```python
from build123d import *

# Parameters (mm, degrees)
SKETCH1_W          = 40
SKETCH1_H          = 30
EXTRUDE1_DEPTH     = 15
SKETCH2_R          = 11
EXTRUDE2_DEPTH     = 10
SKETCH3_R          = 10
EXTRUDE3_DEPTH     = 1
SKETCH4_R          = 17.5
EXTRUDE4_DEPTH     = 8
FILLET1_R          = 2
SKETCH5_OUTSIDE_W  = 56.458
SKETCH5_OUTSIDE_H  = 51.458
SKETCH5_OUTSIDE_R  = 10
CUT_EXTRUDE1_DEPTH = 3


with BuildPart() as part:
    # Sketch1 → Extrude1 (new, symmetric)
    with BuildSketch(Plane(origin=(0, 0, 0), x_dir=(1, 0, 0), z_dir=(0, 1, 0))):
        Rectangle(SKETCH1_W, SKETCH1_H)
    extrude(amount=EXTRUDE1_DEPTH, both=True)

    # Sketch2 → Extrude2 (add)
    with BuildSketch(Plane(origin=(0, 15, 0), x_dir=(1, 0, 0), z_dir=(0, 1, 0))):
        with Locations(Location((0, 0, 0), (0, 0, 270))):
            Circle(SKETCH2_R)
    extrude(amount=EXTRUDE2_DEPTH)

    # Sketch3 → Extrude3 (add)
    with BuildSketch(Plane(origin=(0, 25, 0), x_dir=(1, 0, 0), z_dir=(0, 1, 0))):
        with Locations(Location((0, 0, 0), (0, 0, 270))):
            Circle(SKETCH3_R)
    extrude(amount=EXTRUDE3_DEPTH)

    # Sketch4 → Extrude4 (add)
    with BuildSketch(Plane(origin=(0, 26, 0), x_dir=(1, 0, 0), z_dir=(0, 1, 0))):
        with Locations(Location((0, 0, 0), (0, 0, 270))):
            Circle(SKETCH4_R)
    extrude(amount=EXTRUDE4_DEPTH)

    # Fillet1
    fillet1_edges = [part.edges().sort_by_distance(p)[0] for p in [
        (0, 34, -17.5),
    ]]
    fillet(fillet1_edges, radius=FILLET1_R)

    # Sketch5 outside → Cut-Extrude1 (cut)
    with BuildSketch(Plane(origin=(0, 18, 0), x_dir=(-1, 0, 0), z_dir=(0, 1, 0))):
        Rectangle(SKETCH5_OUTSIDE_W, SKETCH5_OUTSIDE_H)
        with Locations(Location((0, 0, 0), (0, 0, 90))):
            Circle(SKETCH5_OUTSIDE_R, mode=Mode.SUBTRACT)
    extrude(amount=-CUT_EXTRUDE1_DEPTH, mode=Mode.SUBTRACT)


solid = part.part
```
Geometry check sheet. Reference: the model listing, model coordinates, mm. A direction names the side the tool comes from. Round coordinates to 2 decimals unless told otherwise and drop trailing zeros. Loops run counter-clockwise (first coordinate to the right, second up) from the corner with the lowest first, then second, coordinate; pieces in that order, holes last. Notation, with made-up numbers: (-5, 19) - (-1, 19) arc R18 cw to (-1, 36) - close; hole circle Ø1 at (55.5, 55.25). An arc over 180 degrees is marked (long way). Write each question's results on one line, items separated by ' | '. Start each with the question number.
Q1. Gauge pin test, flat ends, axial feed: P1, Ø1.5, axis at y = 23.5, z = 2, coming from the +X side; P2, Ø15, axis at x = -4.5, y = -4.5, coming from the +Z side; P3, Ø4, axis at x = 0.5, y = 18, coming from the +Z side. Record the tip position at first contact, or that the pin passes through.
Q2. Thickness scan on line 1 (Y direction, x = 4.5, z = -9.5); line 2 (Y direction, x = -12.5, z = 3.5); line 3 (Z direction, x = 12, y = -5). Record the ranges inside material, lowest first. Write a range as [from, to].
Q3. Cross-section at A-A on x = 0. Enter the section's corners in (y, z), and give its area (3 significant figures).
Q4. Cross-section at B-B on z = 0. Enter the section's corners in (x, y).
Q5. Cross-section at C-C on y = 23.5. Enter the section's corners in (x, z).
Q6. Release check for a two-part mould opening along Y. For faces 1 (the flat face through (20, 0, 0)), 2 (the flat face through (0, -15, 0)), 3 (the flat face through (-2, 18, -10)) record: +Y half, -Y half, draft (parallel to the pull), parting line (faces both ways), or undercut.
Q7. Cross-section at D-D on y = -7.5. Enter the section's corners in (x, z), and give its area (3 significant figures).
Q8. Access from +Z, -Z, +X, -X, +Y, -Y to the whole of each face (thin tool, end or side, straight path). Record for faces 4 (the flat face through (0, 0, -15)), 5 (the cylindrical face through (-10.648, 28.958, -13.887)), 6 (the cylindrical face through (-10.74, 21.45, -2.38)).
Answers below:
1) P1: stops at x = 10.93 | P2: stops at z = 15 | P3: stops at z = 11
2) line 1: y = [-15, 15], [18, 25], [26, 34] | line 2: y = [-15, 15], [26, 34] | line 3: z = [-15, 15]
3) outline: (-15, -15) - (15, -15) - (15, -10) - (18, -10) - (18, -11) - (25, -11) - (25, -10) - (26, -10) - (26, -17.5) - (32, -17.5) arc R2 ccw to (34, -15.5) - (34, 15.5) arc R2 ccw to (32, 17.5) - (26, 17.5) - (26, 10) - (25, 10) - (25, 11) - (18, 11) - (18, 10) - (15, 10) - (15, 15) - (-15, 15) - close | area: 1,410 mm²
4) outline: (-20, -15) - (20, -15) - (20, 15) - (10, 15) - (10, 18) - (11, 18) - (11, 25) - (10, 25) - (10, 26) - (17.5, 26) - (17.5, 32) arc R2 ccw to (15.5, 34) - (-15.5, 34) arc R2 ccw to (-17.5, 32) - (-17.5, 26) - (-10, 26) - (-10, 25) - (-11, 25) - (-11, 18) - (-10, 18) - (-10, 15) - (-20, 15) - close
5) outline: circle Ø22 at (0, 0)
6) face 1: draft | face 2: -Y half | face 3: undercut
7) outline: (-20, -15) - (20, -15) - (20, 15) - (-20, 15) - close | area: 1,200 mm²
8) face 4: -Z, +X, -X, -Y | face 5: +Y | face 6: none
